Check sheet for the modelled part. Datum: model origin and axes. Units: mm. Round coordinates to 2 decimals unless told otherwise and drop trailing zeros. Order: outer loops, then holes, each group sorted by start corner. A loop starts at its lowest first (then second) coordinate and runs counter-clockwise, first axis right, second up. Notation, with made-up numbers: (78, 77) -> (104, 77) arc R29 cw to (104, 114) -> close; hole circle Ø8 at (30.5, 56.25). An arc over 180 degrees is marked (long way). Answer in a Markdown table with one row per item.
```python
from build123d import *

# Parameters (mm, degrees)
BOSS_EXTRUDE1_DEPTH = 3.5
CUT_EXTRUDE1_REACH  = 34.643
SKETCH2_R           = 3.674588618


with BuildPart() as part:
    # Sketch1 → Boss-Extrude1 (new body)
    with BuildSketch(Plane.XY):
        with BuildLine():
            Line((7.466046977, 5.007712178), (27.067619065, 4.999999613))
            ThreePointArc((27.067619065, 4.999999613), (32.065651345, -0.001967333), (27.063684399, -4.999999613))
            Line((27.063684399, -4.999999613), (7.462112311, -4.992287048))
            ThreePointArc((7.462112311, -4.992287048), (2.464080031, 0.009679898), (7.466046977, 5.007712178))
        make_face()
    extrude(amount=BOSS_EXTRUDE1_DEPTH)

    # Sketch2 → Cut-Extrude1 (cut, up to next)
    with BuildSketch(Plane(origin=(0, 0, 0), x_dir=(-1, 0, 0), z_dir=(0, 0, -1)), mode=Mode.PRIVATE) as cut_extrude1_sk1:
        with Locations((-27.065651732, 0)):
            Circle(SKETCH2_R)
    cut_extrude1_tool1 = extrude(cut_extrude1_sk1.sketch, amount=-CUT_EXTRUDE1_REACH, mode=Mode.PRIVATE) & part.part
    # Sketch2 → Cut-Extrude1 (cut, up to next)
    with BuildSketch(Plane(origin=(0, 0, 0), x_dir=(-1, 0, 0), z_dir=(0, 0, -1)), mode=Mode.PRIVATE) as cut_extrude1_sk2:
        with Locations((-7.464079644, 0.007712565)):
            Circle(SKETCH2_R)
    cut_extrude1_tool2 = extrude(cut_extrude1_sk2.sketch, amount=-CUT_EXTRUDE1_REACH, mode=Mode.PRIVATE) & part.part
    add(cut_extrude1_tool1.solids().sort_by_distance((27.065652, 0, 0))[0], mode=Mode.SUBTRACT)
    add(cut_extrude1_tool2.solids().sort_by_distance((7.46408, 0.007713, 0))[0], mode=Mode.SUBTRACT)


solid = part.part
```
(1) Scan lines: probe 1 along X at (y, z) = (0.5, 3.05); probe 2 along Y at (x, z) = (15.5, 0.4); probe 3 along Y at (x, z) = (29, 2.6). Record each from-to range of solid material in increasing order. Write a range as from..to.
Solutions:
| item | result |
|---|---|
| probe 1 | 2.49..3.82, 11.11..23.43, 30.71..32.04 |
| probe 2 | -5..5 |
| probe 3 | -4.61..-3.12, 3.12..4.61 |
(2) Section check C-C on x = 8. Record the boundary of the cut face in (y, z).
Solutions:
| item | result |
|---|---|
| outline | (-4.99, 0) -> (-3.63, 0) -> (-3.63, 3.5) -> (-4.99, 3.5) -> close; (3.64, 0) -> (5.01, 0) -> (5.01, 3.5) -> (3.64, 3.5) -> close |
(3) Section check D-D on z = 2.8. Record the boundary of the cut face in (x, y).
Solutions:
| item | result |
|---|---|
| outline | (7.46, -4.99) -> (27.06, -5) arc R5 ccw to (27.07, 5) -> (7.47, 5.01) arc R5 ccw to start; hole circle Ø7.35 at (7.46, 0.01); hole circle Ø7.35 at (27.07, 0) |
(4) Section check A-A on x = 23.75. Record the boundary of the cut face in (y, z).
Solutions:
| item | result |
|---|---|
| outline | (-5, 0) -> (-1.58, 0) -> (-1.58, 3.5) -> (-5, 3.5) -> close; (1.58, 0) -> (5, 0) -> (5, 3.5) -> (1.58, 3.5) -> close |
(5) Section check B-B on y = -1. Record the boundary of the cut face in (x, z), plus the area to 3 significant figures.
Solutions:
| item | result |
|---|---|
| outline | (2.57, 0) -> (3.93, 0) -> (3.93, 3.5) -> (2.57, 3.5) -> close; (11, 0) -> (23.53, 0) -> (23.53, 3.5) -> (11, 3.5) -> close; (30.6, 0) -> (31.96, 0) -> (31.96, 3.5) -> (30.6, 3.5) -> close |
| area | 53.4 mm^2 |
(6) Draft check along X on faces 1 (the cylindrical face through (30.737, 0.162, 1.726)), 2 (the flat face through (17, 0, 0)), 3 (the cylindrical face through (11.135, 0.169, 1.726)). Enter one of: pulls with the +X half, pulls with the -X half, needs draft (parallel to the pull), parting line crosses it, or undercut.
Solutions:
| item | result |
|---|---|
| face 1 | undercut |
| face 2 | needs draft |
| face 3 | undercut |
